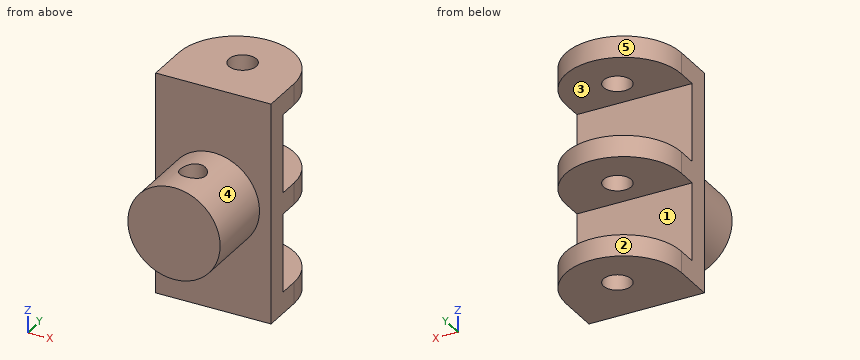
```python
from build123d import *

# Parameters (mm, degrees)
SKETCH1_R               = 12
BOSS_EXTRUDE1_DEPTH     = 191.5
SKETCH2_R               = 40
BOSS_EXTRUDE2_DEPTH     = 62
SKETCH3_W               = 68
SKETCH3_H               = 67
CUT_EXTRUDE5_DEPTH      = 233.52580502
CUT_EXTRUDE8_DEPTH      = 233.52580502
CUT_EXTRUDE8_DEPTH_BACK = 233.52580502
SKETCH4_R               = 11


with BuildPart() as part:
    # Sketch1 → Boss-Extrude1 (new body)
    with BuildSketch(Plane.XY):
        with BuildLine():
            Line((0, 0), (0, 36))
            ThreePointArc((0, 36), (50, 86), (100, 36))
            Line((100, 36), (100, 0))
            Line((100, 0), (0, 0))
        make_face()
        with Locations((50, 46)):
            Circle(SKETCH1_R, mode=Mode.SUBTRACT)
    extrude(amount=BOSS_EXTRUDE1_DEPTH)

    # Sketch2 → Boss-Extrude2 (add)
    with BuildSketch(Plane(origin=(0, 0, 0), x_dir=(-1, 0, 0), z_dir=(0, -1, 0))):
        with Locations(Location((-50, -95.75, 0), (0, 0, 180))):
            Circle(SKETCH2_R)
    extrude(amount=BOSS_EXTRUDE2_DEPTH)

    # Sketch3 → Cut-Extrude5 (cut, through all)
    with BuildSketch(Plane(origin=(0, 0, 0), x_dir=(0, 0, -1), z_dir=(1, 0, 0))):
        with Locations((-52.5, 52.5)):
            Rectangle(SKETCH3_W, SKETCH3_H)
        with Locations((-139, 52.5)):
            Rectangle(SKETCH3_W, SKETCH3_H)
    extrude(amount=CUT_EXTRUDE5_DEPTH, mode=Mode.SUBTRACT)

    # Sketch4 → Cut-Extrude8 (cut, two sides: drawn at the far end of the back side and taken through both)
    with BuildSketch(Plane.XY.offset(-CUT_EXTRUDE8_DEPTH_BACK)):
        with Locations((50, -32)):
            Circle(SKETCH4_R)
    extrude(amount=CUT_EXTRUDE8_DEPTH + CUT_EXTRUDE8_DEPTH_BACK, mode=Mode.SUBTRACT)


solid = part.part
```
Work out the finished part from the listing and answer in its coordinate system (mm). Face numbers are marked on the shaded views. A direction names the side the tool comes from. Give positions to 0.01 mm unless a question says otherwise; leave off trailing zeros. Loops run counter-clockwise (first coordinate to the right, second up) from the corner with the lowest first, then second, coordinate; pieces in that order, holes last. Notation, with made-up numbers: M 3,78 L 13,78 A16 ccw 13,107 Z; hole C 47.5,44.25 d10. An arc over 180 degrees is marked long. One line per item, written item: value. Start each with the question number.
1. Find section A-A (x = 50). State how many separate pieces and enclosed holes the cut face has, and give its area (4 significant figures).
2. Find section D-D (y = 41.5). Give the vertices of the cut face in (x, z), and give its area (3 significant figures).
3. Each of these flat-tipped pins is pushed along its axis until it touches: P1, Ø1, axis at x = 80, z = 86.5, coming from the +Y side; P2, Ø1, axis at y = -33, z = 91, coming from the +X side; P3, Ø20.5, axis at x = 40.5, z = 148.5, coming from the +Y side. Where does it stop, or does it pass through?
4. Find section C-C (y = 74). Give the vertices of the cut face in (x, z).
5. Find section B-B (z = 95.75). Give the vertices of the cut face in (x, y), and give its area (3 significant figures).
6. Determine the mould class of the marked faces 3, 4 and 5 for opening direction Z: released by +Z, released by -Z, zero draft, split by the parting line, or undercut.
7. Which of the six approach directions +Z, -Z, +X, -X, +Y, -Y give full straight-line access (tool end or side, diameter ignored) to the marked faces 1 and 2?
8. Find the intervals of material crossed by probe 1 along Z at (x, y) = (35, 69); probe 2 along Y at (x, z) = (50, 92.5); probe 3 along Y at (x, z) = (50, 184), in increasing order.
Reported:
1. separate pieces: 5
1. enclosed holes: 0
1. area: 9,225 mm²
2. outline: M 0.3,0 L 38.88,0 L 38.88,18.5 L 0.3,18.5 Z; M 0.3,86.5 L 38.88,86.5 L 38.88,105 L 0.3,105 Z; M 0.3,173 L 38.88,173 L 38.88,191.5 L 0.3,191.5 Z; M 61.12,0 L 99.7,0 L 99.7,18.5 L 61.12,18.5 Z; M 61.12,86.5 L 99.7,86.5 L 99.7,105 L 61.12,105 Z; M 61.12,173 L 99.7,173 L 99.7,191.5 L 61.12,191.5 Z
2. area: 4,280 mm²
3. P1: stops at y = 76.37
3. P2: stops at x = 89.77
3. P3: stops at y = 19
4. outline: M 17.5,0 L 82.5,0 L 82.5,18.5 L 17.5,18.5 Z; M 17.5,86.5 L 82.5,86.5 L 82.5,105 L 17.5,105 Z; M 17.5,173 L 82.5,173 L 82.5,191.5 L 17.5,191.5 Z
5. outline: M 0,0 L 10,0 L 10,-62 L 90,-62 L 90,0 L 100,0 L 100,36 A50 ccw 0,36 Z; hole C 50,46 d24; hole C 50,-32 d22
5. area: 11,700 mm²
6. face 3: undercut
6. face 4: split by the parting line
6. face 5: zero draft
7. face 1: +X, -X, +Y
7. face 2: +Z, -Z, +Y
8. probe 1: z = 0 to 18.5, 86.5 to 105, 173 to 191.5
8. probe 2: y = -62 to -43, -21 to 34, 58 to 86
8. probe 3: y = 0 to 34, 58 to 86
